Verification items for this drawing (mm, ordinates from the low corner). A direction names the side the tool comes from. Round coordinates to 2 decimals unless told otherwise and drop trailing zeros. Order: outer loops, then holes, each group sorted by start corner. A loop starts at its lowest first (then second) coordinate and runs counter-clockwise, first axis right, second up. Notation, with made-up numbers: (29.25, -15) -> (65.25, -15) arc R10 cw to (65.25, -1) -> close; hole circle Ø6 at (21, -37). An arc over 180 degrees is marked (long way). Answer in a Markdown table with one row per item. Add a question column.
1. Sectioned sample at B-B, the plane x = 60. Record the boundary of the cut face in (y, z), then the cut area to 3 significant figures.
2. Sectioned sample at C-C, the plane z = 52.5. Record the boundary of the cut face in (x, y).
3. Access from +Z, -Z, +X, -X, +Y, -Y to the whole of each face (thin tool, end or side, straight path). Record for the marked faces 4 and 5.
4. Material ranges on L1, parallel to X at y = 5, z = 20; L2, parallel to Y at x = 39.5, z = 13, recorded low to high. Write a range as from..to.
5. Sectioned sample at A-A, the plane z = 20. Record the boundary of the cut face in (x, y), then the cut area to 4 significant figures.
6. Depth check by flat-ended pin: P1, Ø18.5, axis at x = 60, z = 70, coming from the +Y side; P2, Ø10, axis at y = 89.5, z = 28, coming from the +X side; P3, Ø8, axis at x = 66, z = 10, coming from the -Y side. Enter the tip coordinate at first touch or a pass-through.
7. Draft check along X on the marked faces 1, 2 and 3. Enter one of: +X half, -X half, draft (parallel to the pull), parting line (faces both ways), or undercut.
8. Sectioned sample at D-D, the plane y = 79. Record the boundary of the cut face in (x, z), then the cut area to 3 significant figures.
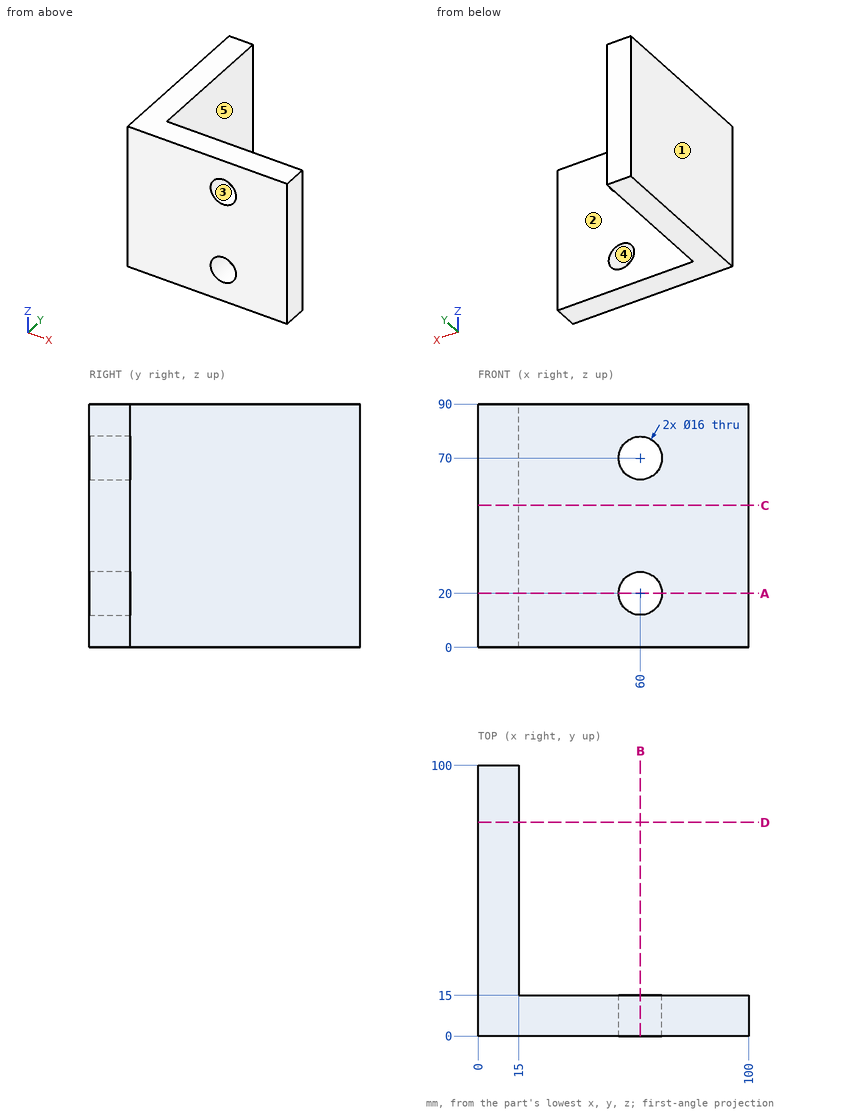
Answer key:
| question | item | result |
|---|---|---|
| 1 | outline | (0, 0) -> (15, 0) -> (15, 12) -> (0, 12) -> close; (0, 28) -> (15, 28) -> (15, 62) -> (0, 62) -> close; (0, 78) -> (15, 78) -> (15, 90) -> (0, 90) -> close |
| 1 | area | 870 mm² |
| 2 | outline | (0, 0) -> (100, 0) -> (100, 15) -> (15, 15) -> (15, 100) -> (0, 100) -> close |
| 3 | face 4 | +Y, -Y |
| 3 | face 5 | +Z, -Z, +X, +Y |
| 4 | L1 | x = 0..52, 68..100 |
| 4 | L2 | y = 0..15 |
| 5 | outline | (0, 0) -> (52, 0) -> (52, 15) -> (15, 15) -> (15, 100) -> (0, 100) -> close; (68, 0) -> (100, 0) -> (100, 15) -> (68, 15) -> close |
| 5 | area | 2,535 mm² |
| 6 | P1 | stops at y = 15 |
| 6 | P2 | stops at x = 15 |
| 6 | P3 | stops at y = 0 |
| 7 | face 1 | -X half |
| 7 | face 2 | draft |
| 7 | face 3 | undercut |
| 8 | outline | (0, 0) -> (15, 0) -> (15, 90) -> (0, 90) -> close |
| 8 | area | 1,350 mm² |
